from build123d import *

# Parameters (mm, degrees)
SKETCH1_W           = 300
SKETCH1_H           = 200
BOSS_EXTRUDE1_DEPTH = 20
SKETCH2_W           = 270
SKETCH2_H           = 160
CUT_EXTRUDE1_DEPTH  = 10
SKETCH3_R           = 30
CUT_EXTRUDE2_DEPTH  = 6


with BuildPart() as part:
    # Sketch1 → Boss-Extrude1 (new body)
    with BuildSketch(Plane.XY):
        Rectangle(SKETCH1_W, SKETCH1_H)
    extrude(amount=BOSS_EXTRUDE1_DEPTH)

    # Sketch2 → Cut-Extrude1 (cut)
    with BuildSketch(Plane(origin=(0, 0, 0), x_dir=(-1, 0, 0), z_dir=(0, 0, -1))):
        Rectangle(SKETCH2_W, SKETCH2_H)
    extrude(amount=-CUT_EXTRUDE1_DEPTH, mode=Mode.SUBTRACT)

    # Sketch3 → Cut-Extrude2 (cut)
    with BuildSketch(Plane(origin=(0, 0, 10), x_dir=(-1, 0, 0), z_dir=(0, 0, -1))):
        Circle(SKETCH3_R)
    extrude(amount=-CUT_EXTRUDE2_DEPTH, mode=Mode.SUBTRACT)


solid = part.part
Model file for the job. Use its own axes, mm. A direction names the side the tool comes from. Give positions to 0.01 mm unless a question says otherwise; leave off trailing zeros. Write each loop counter-clockwise with the first axis right and the second up, starting at its lowest first coordinate (ties: lowest second). Pieces come first, ordered by that corner, then holes. Notation, with made-up numbers: (-2.5, 42.25) - (48.5, 42.25) arc R6 ccw to (48.5, 47.25) - close; hole circle Ø5 at (36.5, 46.5). An arc over 180 degrees is marked (long way). Answer as CSV lines item,"result".
1. Two-plate mould, pull along Y, no slides. Class faces 1 (the face through (-150, -1, 10)), 2 (the face through (-2, -100, 10)), 3 (the face through (-135, -1, 5)): +Y half, -Y half, draft (parallel to the pull), parting line (faces both ways), or undercut.
Responses:
face 1,"draft"
face 2,"-Y half"
face 3,"undercut"
2. 3-axis set-ups, long thin cutter, end or side, ignore diameter. For faces 4 (the face through (150, -1, 10)), 5 (the face through (135, -1, 5)): which of +Z, -Z, +X, -X, +Y, -Y reach the whole face in a straight line?
Responses:
face 4,"+Z, -Z, +X, +Y, -Y"
face 5,"-Z"
3. Band-saw the part on C-C (y = -76). Write the cut outline in (x, z), and give its area (3 significant figures).
Responses:
outline,"(-150, 0) - (-135, 0) - (-135, 10) - (135, 10) - (135, 0) - (150, 0) - (150, 20) - (-150, 20) - close"
area,"3,300 mm2"
4. Band-saw the part on B-B (y = 0). Write the cut outline in (x, z).
Responses:
outline,"(-150, 0) - (-135, 0) - (-135, 10) - (-30, 10) - (-30, 16) - (30, 16) - (30, 10) - (135, 10) - (135, 0) - (150, 0) - (150, 20) - (-150, 20) - close"
5. Band-saw the part on D-D (x = 0). Write the cut outline in (y, z), and give its area (3 significant figures).
Responses:
outline,"(-100, 0) - (-80, 0) - (-80, 10) - (-30, 10) - (-30, 16) - (30, 16) - (30, 10) - (80, 10) - (80, 0) - (100, 0) - (100, 20) - (-100, 20) - close"
area,"2,040 mm2"
6. Pin check, flat tip, straight feed: pin 1 (4 mm diameter, centred on x = 61, y = 0.5, fed in from -Z). Stop position of the tip, or through.
Responses:
pin 1,"stops at z = 10"
7. Drill centre lines: L1, parallel to Y at x = -120, z = 5.25; L2, parallel to Y at x = 0, z = 14.8; L3, parallel to X at y = -61, z = 6.25. Where is each one in solid material? Low to high. Write a range as [from, to].
Responses:
L1,"y = [-100, -80], [80, 100]"
L2,"y = [-100, -30], [30, 100]"
L3,"x = [-150, -135], [135, 150]"
8. Band-saw the part on A-A (x = -130). Write the cut outline in (y, z).
Responses:
outline,"(-100, 0) - (-80, 0) - (-80, 10) - (80, 10) - (80, 0) - (100, 0) - (100, 20) - (-100, 20) - close"
